from build123d import *

# Parameters (mm, degrees)
BOSS_EXTRUDE1_DEPTH = 4


with BuildPart() as part:
    # Sketch1 → Boss-Extrude1 (new body)
    with BuildSketch(Plane(origin=(0, 0, 0), x_dir=(0, 0, -1), z_dir=(1, 0, 0))):
        Polygon((-9.5, 5.484827557), (-9.5, -5.484827557), (0, -10.969655115), (9.5, -5.484827557), (9.5, 5.484827557), (0, 10.969655115), align=None)
    extrude(amount=BOSS_EXTRUDE1_DEPTH)

    # Sketch2 → Cut-Revolve1 (revolve, cut)
    with BuildSketch(Plane.XY):
        Polygon((0, 13.95), (0, 9.5), (2, 12.964101615), (4, 9.5), (4, 13.95), align=None)
    revolve(axis=Axis((50, 0, 0), (-1, 0, 0)), mode=Mode.SUBTRACT)

    # Sketch3 → Cut-Revolve2 (revolve, cut)
    with BuildSketch(Plane.XY, mode=Mode.PRIVATE) as cut_revolve2_sk:
        Polygon((0, 0), (0, 7), (0.5415, 6.4585), (3.4585, 6.4585), (4, 7), (4, 0), align=None)
    revolve(cut_revolve2_sk.sketch.rotate(Axis((4, 0, 0), (-1, 0, 0)), 90), axis=Axis((4, 0, 0), (-1, 0, 0)), mode=Mode.SUBTRACT)


solid = part.part
Source: CAD feature listing. Evaluate the final solid. Frame: model axes, mm. Give positions to 0.01 mm unless a question says otherwise; leave off trailing zeros. Order: outer loops, then holes, each group sorted by start corner. A loop starts at its lowest first (then second) coordinate and runs counter-clockwise, first axis right, second up. Notation, with made-up numbers: (24.25, 86.5) -> (77.25, 86.5) arc R11 ccw to (77.25, 107.5) -> close; hole circle Ø3 at (83, -19). An arc over 180 degrees is marked (long way). Write item = value, one per line.
Q1. Material intervals for line 1 (Z direction, x = 1.5, y = 1.25); line 2 (Z direction, x = 2.8, y = 5.5); line 3 (Y direction, x = 1.25, z = 1.75), sorted ascending. Write a range as from..to.
Data:
line_1 = -9.5..-6.34, 6.34..9.5
line_2 = -9.47..-3.39, 3.39..9.47
line_3 = -9.96..-6.22, 6.22..9.96
Q2. Cut plane A-A, the plane x = 2.8. Output: boundary loops of the cut face in (y, z), and give its area (3 significant figures).
Data:
outline = (-10.97, 0) -> (-5.48, -9.5) -> (5.48, -9.5) -> (10.97, 0) -> (5.48, 9.5) -> (-5.48, 9.5) -> close; hole circle Ø12.92 at (0, 0)
area = 182 mm^2
Q3. Pull-direction query (Y, two-part tool) for faces 1 (the face through (4, -6, 4)), 2 (the face through (2.02, -6.404, 0.841)), 3 (the face through (0.206, 4.908, 8.549)), 4 (the face through (3.798, -4.946, 8.519)); classes: released by +Y, released by -Y, zero draft, split by the parting line, or undercut.
Data:
face_1 = zero draft
face_2 = undercut
face_3 = released by +Y
face_4 = released by -Y
